from build123d import *

# Parameters (mm, degrees)
SKETCH1_W           = 10
SKETCH1_H           = 3.75
BOSS_EXTRUDE1_DEPTH = 18
SKETCH2_R           = 1.75
CUT_EXTRUDE1_DEPTH  = 20
SKETCH3_W           = 10
SKETCH3_H           = 12
BOSS_EXTRUDE2_DEPTH = 5
CUT_EXTRUDE2_DEPTH  = 10
CHAMFER1_SIZE       = 1
CUT_EXTRUDE3_DEPTH  = 10


with BuildPart() as part:
    # Sketch1 → Boss-Extrude1 (new body)
    with BuildSketch(Plane(origin=(0, 0, 0), x_dir=(1, 0, 0), z_dir=(0, 1, 0))):
        with Locations((5, 1.875)):
            Rectangle(SKETCH1_W, SKETCH1_H)
    extrude(amount=BOSS_EXTRUDE1_DEPTH)

    # Sketch2 → Cut-Extrude1 (cut)
    with BuildSketch(Plane.XY):
        with Locations((5, 12.7)):
            Circle(SKETCH2_R)
    extrude(amount=-CUT_EXTRUDE1_DEPTH, mode=Mode.SUBTRACT)

    # Sketch3 → Boss-Extrude2 (add)
    with BuildSketch(Plane.XZ):
        with Locations((5, 6)):
            Rectangle(SKETCH3_W, SKETCH3_H)
    extrude(amount=-BOSS_EXTRUDE2_DEPTH)

    # Sketch4 → Cut-Extrude2 (cut)
    with BuildSketch(Plane(origin=(0, 5, 0), x_dir=(1, 0, 0), z_dir=(0, 1, 0))):
        with BuildLine():
            Line((3.5, -10.25), (6.5, -10.25))
            ThreePointArc((6.5, -10.25), (8.75, -8), (6.5, -5.75))
            Line((6.5, -5.75), (3.5, -5.75))
            ThreePointArc((3.5, -5.75), (1.25, -8), (3.5, -10.25))
        make_face()
    extrude(amount=-CUT_EXTRUDE2_DEPTH, mode=Mode.SUBTRACT)

    # Chamfer1
    chamfer1_edges = [part.edges().sort_by_distance(p)[0] for p in [
        (10, 18, -1.875),
        (0, 2.5, 12),
        (10, 2.5, 12),
        (0, 18, -1.875),
        (5, 0, -3.75),
    ]]
    chamfer(chamfer1_edges, length=CHAMFER1_SIZE)

    # Sketch5 → Cut-Extrude3 (cut)
    with BuildSketch(Plane.XY):
        with BuildLine():
            Line((6.75, 14.45), (6.75, 10.95))
            ThreePointArc((6.75, 10.95), (5, 9.2), (3.25, 10.95))
            Line((3.25, 10.95), (3.25, 14.45))
            ThreePointArc((3.25, 14.45), (5, 16.2), (6.75, 14.45))
        make_face()
    extrude(amount=-CUT_EXTRUDE3_DEPTH, mode=Mode.SUBTRACT)


solid = part.part
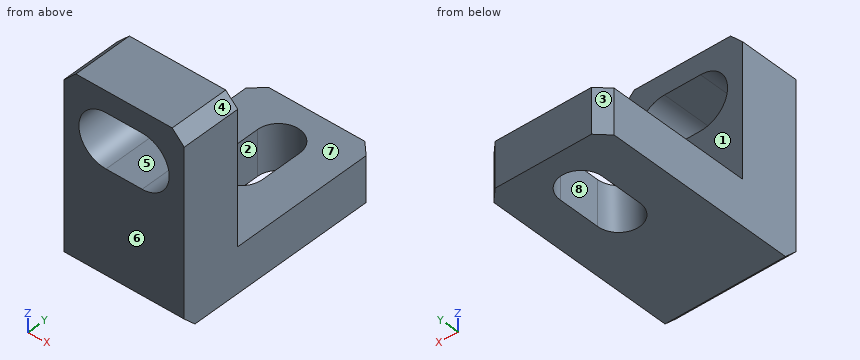
Could you check a few things on this model? Use its own coordinates, in mm. Face numbers are marked on the shaded views. A direction names the side the tool comes from. Round coordinates to 2 decimals unless told otherwise and drop trailing zeros. Order: outer loops, then holes, each group sorted by start corner. A loop starts at its lowest first (then second) coordinate and runs counter-clockwise, first axis right, second up. Notation, with made-up numbers: M 79.5,25.5 L 105.5,25.5 A20 ccw 105.5,33.5 Z; hole C 44,77.25 d3. An arc over 180 degrees is marked long. One line per item, written item: value.
(1) I need wall thicknesses on line 1 along Y through (x, z) = (7, 5.75); line 2 along Z through (x, y) = (5.75, 7). Which ranges of each line are inside material? Lowest first, please. Write a range as from..to.
Ans:
line 1: y = 0..5
line 2: z = -3.75..0
(2) I'm going to push flat-ended pins straight in: P1, Ø1, axis at y = 7, z = 5.5, coming from the +X side; P2, Ø5, axis at x = 3, y = 14.5, coming from the +Z side. Where does each tip first touch, or does it pass through?
Ans:
P1: passes through
P2: stops at z = 0
(3) Imagine slicing it at A-A (z = 8). Write out the boundary of the cut face in (x, y), and give its area (3 significant figures).
Ans:
outline: M 0,0 L 1.25,0 L 1.25,5 L 0,5 Z; M 8.75,0 L 10,0 L 10,5 L 8.75,5 Z
area: 12.5 mm^2
(4) If we mould it in two halves opening along X, with no side actions, what happens to the marked faces 1, 2, 3 and 4? For each: released by +X, released by -X, zero draft, split by the parting line, or undercut.
Ans:
face 1: zero draft
face 2: undercut
face 3: released by -X
face 4: released by +X
(5) Which directions (+Z, -Z, +X, -X, +Y, -Y) give clear straight access to the entire face, cutting with the end or side of a thin tool? Please do the marked faces 5, 6, 7 and 8.
Ans:
face 5: +Y, -Y
face 6: +Z, -Z, +X, -X, -Y
face 7: +Z, +X, -X, +Y
face 8: +Z, -Z
(6) Imagine slicing it at D-D (y = 11.5). Write out the boundary of the cut face in (x, z).
Ans:
outline: M 0,-3.75 L 3.25,-3.75 L 3.25,0 L 0,0 Z; M 6.75,-3.75 L 10,-3.75 L 10,0 L 6.75,0 Z
(7) Imagine slicing it at C-C (x = 5). Write out the boundary of the cut face in (y, z), and give its area (4 significant figures).
Ans:
outline: M 0,-2.75 L 1,-3.75 L 9.2,-3.75 L 9.2,0 L 5,0 L 5,5.75 L 0,5.75 Z; M 0,10.25 L 5,10.25 L 5,12 L 0,12 Z; M 16.2,-3.75 L 18,-3.75 L 18,0 L 16.2,0 Z
area: 78.25 mm^2
(8) Imagine slicing it at B-B (y = 3.75). Write out the boundary of the cut face in (x, z), and give its area (3 significant figures).
Ans:
outline: M 0,-3.75 L 10,-3.75 L 10,11 L 9,12 L 1,12 L 0,11 Z; hole M 3.5,5.75 L 6.5,5.75 A2.25 ccw 6.5,10.25 L 3.5,10.25 A2.25 ccw Z
area: 127 mm^2
